from build123d import *
from OCP.BRepFilletAPI import BRepFilletAPI_MakeChamfer

# Parameters (mm, degrees)
CHAMFER1_SIZE  = 0.5
CHAMFER1_SIZE2 = 0.512980744


with BuildPart() as part:
    # Sketch1 → Revolve1 (revolve)
    with BuildSketch(Plane.XY, mode=Mode.PRIVATE) as revolve1_sk:
        Polygon((8.25, 35), (23, 35), (23.5, 15), (23.5, 10), (40, 10), (40, 0), (8.25, 0), align=None)
    revolve(revolve1_sk.sketch.rotate(Axis((0, 0, 0), (0, 1, 0)), 90), axis=Axis((0, 0, 0), (0, 1, 0)))

    # Chamfer1: one chamfer whose edges measure the first distance from different faces: ONE call of the kernel's chamfer builder (chamfer() names one face for all edges)
    chamfer1_edges_1 = [part.edges().sort_by_distance(p)[0] for p in [
        (0, 10, 40),
        (0, 0, 40),
        (0, 0, 8.25),
        (0, 35, 8.25),
    ]]
    chamfer1_edges_2 = [part.edges().sort_by_distance(p)[0] for p in [
        (0, 35, 23),
    ]]
    chamfer1_side_2 = [part.faces().sort_by_distance(p)[0] for p in [
        (0, 35, 8.900538239),
    ]]
    chamfer1 = BRepFilletAPI_MakeChamfer(part.part.solid().wrapped)
    for e in chamfer1_edges_1:
        chamfer1.Add(CHAMFER1_SIZE, e.wrapped)
    for e in chamfer1_edges_2:
        chamfer1.Add(CHAMFER1_SIZE, CHAMFER1_SIZE2, e.wrapped, chamfer1_side_2[0].wrapped)  # the first distance lies on this face
    add(Compound.cast(chamfer1.Shape()), mode=Mode.REPLACE)


solid = part.part
Work out the finished part from the listing and answer in its coordinate system (mm). A direction names the side the tool comes from. Give positions to 0.01 mm unless a question says otherwise; leave off trailing zeros. Write each loop counter-clockwise with the first axis right and the second up, starting at its lowest first coordinate (ties: lowest second). Pieces come first, ordered by that corner, then holes. Notation, with made-up numbers: M 52,3 L 98,3 A27 cw 98,33 Z; hole C 42,5 d11. An arc over 180 degrees is marked long. Answer as CSV lines item,"result".
Q1. Find the intervals of material crossed by probe 1 along X at (y, z) = (14.5, 0); probe 2 along X at (y, z) = (8, 0); probe 3 along Y at (x, z) = (-15, -32), in increasing order. Write a range as [from, to].
A:
probe 1,"x = [-23.5, -8.25], [8.25, 23.5]"
probe 2,"x = [-40, -8.25], [8.25, 40]"
probe 3,"y = [0, 10]"
Q2. A cutting plane is placed at D-D on y = 28. Write down the section's boundary in (x, z) (3 decimals), plus the area to 3 significant figures.
A:
outline,"C 0,0 d46.35; hole C 0,0 d16.5"
area,"1,470 mm²"
Q3. A tool of negligible diameter and unlimited length cuts with its end or side. For faces 1 (the cylindrical face through (-1.76, 4.94, 39.96)), 2 (the flat face through (17, 10, 17)), from which of +Z, -Z, +X, -X, +Y, -Y can it reach the whole face along a straight path? Write none if from no direction.
A:
face 1,"+Y, -Y"
face 2,"+Y"
Q4. A cutting plane is placed at C-C on y = 21. Write down the section's boundary in (x, z).
A:
outline,"C 0,0 d46.7; hole C 0,0 d16.5"
Q5. A cutting plane is placed at A-A on z = 0. Write down the section's boundary in (x, y), plus the area to 3 significant figures.
A:
outline,"M -40,0.5 L -39.5,0 L -8.75,0 L -8.25,0.5 L -8.25,34.5 L -8.75,35 L -22.5,35 L -23.01,34.49 L -23.5,15 L -23.5,10 L -39.5,10 L -40,9.5 Z; M 8.25,0.5 L 8.75,0 L 39.5,0 L 40,0.5 L 40,9.5 L 39.5,10 L 23.5,10 L 23.5,15 L 23.01,34.49 L 22.5,35 L 8.75,35 L 8.25,34.5 Z"
area,"1,390 mm²"
Q6. Given P1, Ø3, axis at x = 19, y = 27.5, coming from the -Z side; P2, Ø5, axis at y = 10, z = 10.5, coming from the -X side; P3, Ø3, axis at x = 9.5, z = -29, coming from the +Y side, each flat-ended and moving along its own axis, determine where each tip first touches the part or whether it passes through.
A:
P1,"stops at z = -15.21"
P2,"stops at x = -39.18"
P3,"stops at y = 10"
Q7. The mould has two halves that part along Z. Classify faces 3 (the cylindrical face through (-23.3, 12.46, 3.06)), 4 (the flat face through (-9, 0, 1)), 5 (the cylindrical face through (-2.48, 17.74, -7.87)): +Z half, -Z half, draft (parallel to the pull), parting line (faces both ways), or undercut.
A:
face 3,"parting line"
face 4,"draft"
face 5,"undercut"
Q8. A cutting plane is placed at B-B on x = 0. Write down the section's boundary in (y, z), plus the area to 3 significant figures.
A:
outline,"M 0,-39.5 L 0.5,-40 L 9.5,-40 L 10,-39.5 L 10,-23.5 L 15,-23.5 L 34.49,-23.01 L 35,-22.5 L 35,-8.75 L 34.5,-8.25 L 0.5,-8.25 L 0,-8.75 Z; M 0,8.75 L 0.5,8.25 L 34.5,8.25 L 35,8.75 L 35,22.5 L 34.49,23.01 L 15,23.5 L 10,23.5 L 10,39.5 L 9.5,40 L 0.5,40 L 0,39.5 Z"
area,"1,390 mm²"
